from build123d import *

# Parameters (mm, degrees)
SKETCH_2_W          = 7.7
SKETCH_2_H          = 1
CUT_EXTRUDE_1_DEPTH = 2
FILLET_1_R          = 0.4


with BuildPart() as part:
    # 草图1 → 旋转1 (revolve)
    with BuildSketch(Plane.XY):
        with BuildLine():
            Line((3, 3.85), (3, 2))
            Line((3, 2), (7, 2))
            Line((7, 2), (15, 2))
            Line((15, 2), (15, 0))
            Line((15, 0), (0, 0))
            ThreePointArc((0, 0), (0.838550848, 2.440414924), (3, 3.85))
        make_face()
    revolve(axis=Axis((0, 0, 0), (1, 0, 0)))

    # 草图2 → 切除-拉伸1 (cut)
    with BuildSketch(Plane(origin=(0, 0, 0), x_dir=(0, 0, -1), z_dir=(1, 0, 0))):
        Rectangle(SKETCH_2_W, SKETCH_2_H)
    extrude(amount=CUT_EXTRUDE_1_DEPTH, mode=Mode.SUBTRACT)

    # 圆角1
    fillet_1_edges = [part.edges().sort_by_distance(p)[0] for p in [
        (3, -2, 0),
    ]]
    fillet(fillet_1_edges, radius=FILLET_1_R)


solid = part.part
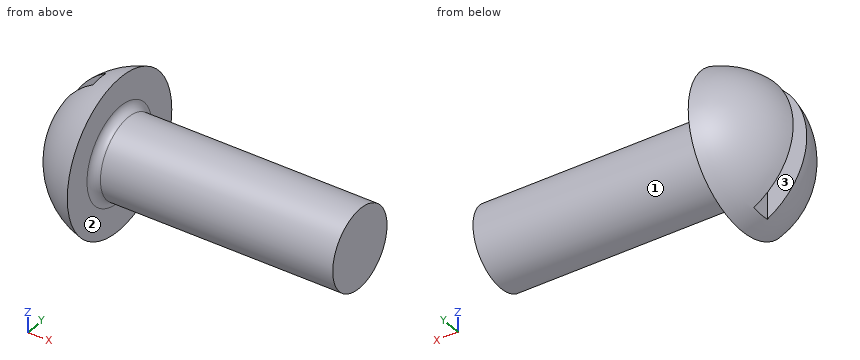
Check sheet for the modelled part. Datum: model origin and axes. Units: mm. Face numbers are marked on the shaded views. Give positions to 0.01 mm unless a question says otherwise; leave off trailing zeros. Write each loop counter-clockwise with the first axis right and the second up, starting at its lowest first coordinate (ties: lowest second). Pieces come first, ordered by that corner, then holes. Notation, with made-up numbers: (23, -36.5) -> (43, -36.5) arc R26 cw to (43, 2.5) -> close; hole circle Ø6 at (1, 23.25). An arc over 180 degrees is marked (long way). One line per item, written item: value. Start each with the question number.
Item 1: Section check A-A on y = 0. Record the cut outline in (x, z).
Item 2: Section check C-C on x = 8. Record the cut outline in (y, z), then the cut area to 3 significant figures.
Item 3: Section check D-D on z = -2.75. Record the cut outline in (x, y), then the cut area to 3 significant figures.
Item 4: Material ranges on probe 1 along X at (y, z) = (0, -3); probe 2 along X at (y, z) = (-2.25, -2.5); probe 3 along Z at (x, y) = (5.25, -0.25), recorded low to high. Write a range as from..to.
Item 5: Draft check along Y on the marked faces 1, 2 and 3. Enter one of: +Y half, -Y half, draft (parallel to the pull), parting line (faces both ways), or undercut.
Item 6: Section check B-B on z = 0. Record the cut outline in (x, y), then the cut area to 3 significant figures.
Item 7: Gauge pin test, flat ends, axial feed: pin 1 (3 mm diameter, centred on x = 9, y = -1.5, fed in from +Z); pin 2 (2 mm diameter, centred on x = 13, z = -1, fed in from +Y); pin 3 (1 mm diameter, centred on x = 1, z = -1, fed in from +Y). Record the tip position at first contact, or that the pin passes through.
Results list:
1. outline: (2, -3.45) arc R3.97 ccw to (3, -3.85) -> (3, -2.4) arc R0.4 cw to (3.4, -2) -> (15, -2) -> (15, 2) -> (3.4, 2) arc R0.4 cw to (3, 2.4) -> (3, 3.85) arc R3.97 ccw to (2, 3.45) -> close
2. outline: circle Ø4 at (0, 0)
2. area: 12.6 mm²
3. outline: (1.15, -0.5) arc R2.86 ccw to (3, -2.69) -> (3, 2.69) arc R2.86 ccw to (1.15, 0.5) -> (2, 0.5) -> (2, -0.5) -> close
3. area: 6.55 mm²
4. probe 1: 2..3
4. probe 2: 1.86..3
4. probe 3: -1.98..1.98
5. face 1: parting line
5. face 2: draft
5. face 3: undercut
6. outline: (0.03, -0.5) arc R3.97 ccw to (3, -3.85) -> (3, -2.4) arc R0.4 cw to (3.4, -2) -> (15, -2) -> (15, 2) -> (3.4, 2) arc R0.4 cw to (3, 2.4) -> (3, 3.85) arc R3.97 ccw to (0.03, 0.5) -> (2, 0.5) -> (2, -0.5) -> close
6. area: 63.2 mm²
7. pin 1: z = 2
7. pin 2: y = 2
7. pin 3: y = 2.97
